For this review, take the finished solid that the model builds, in its own axes (mm). Face numbers are marked on the shaded views. A direction names the side the tool comes from. Round coordinates to 2 decimals unless told otherwise and drop trailing zeros. Write each loop counter-clockwise with the first axis right and the second up, starting at its lowest first coordinate (ties: lowest second). Pieces come first, ordered by that corner, then holes.
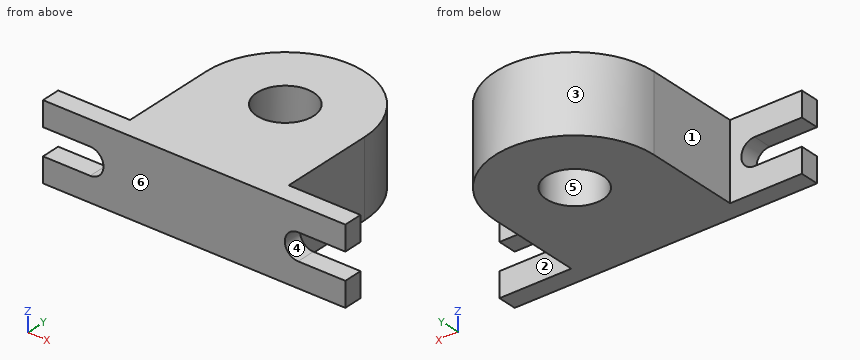
from build123d import *

# Parameters (mm, degrees)
SKETCH_1_R          = 7.5
EXTRUDE_1_DEPTH     = 20
CUT_EXTRUDE_1_DEPTH = 65.156059729


with BuildPart() as part:
    # 草图1 → 凸台-拉伸1 (new body)
    with BuildSketch(Plane.XY):
        with BuildLine():
            Line((21, 0), (21, -25))
            Line((21, -25), (40, -25))
            Line((40, -25), (40, -30))
            Line((40, -30), (21, -30))
            Line((21, -30), (-21, -30))
            Line((-21, -30), (-40, -30))
            Line((-40, -30), (-40, -25))
            Line((-40, -25), (-21, -25))
            Line((-21, -25), (-21, 0))
            ThreePointArc((-21, 0), (0, 21), (21, 0))
        make_face()
        Circle(SKETCH_1_R, mode=Mode.SUBTRACT)
    extrude(amount=EXTRUDE_1_DEPTH)

    # 草图2 → 切除-拉伸1 (cut, through all)
    with BuildSketch(Plane(origin=(0, -25, 0), x_dir=(1, 0, 0), z_dir=(0, 1, 0))):
        with BuildLine():
            Line((-27.5, -6.5), (-40, -6.5))
            Line((-40, -6.5), (-40, -13.5))
            Line((-40, -13.5), (-27.5, -13.5))
            ThreePointArc((-27.5, -13.5), (-24, -10), (-27.5, -6.5))
        make_face()
        with BuildLine():
            Line((40, -13.5), (27.5, -13.5))
            ThreePointArc((27.5, -13.5), (24, -10), (27.5, -6.5))
            Line((27.5, -6.5), (40, -6.5))
            Line((40, -6.5), (40, -13.5))
        make_face()
    extrude(amount=-CUT_EXTRUDE_1_DEPTH, mode=Mode.SUBTRACT)


solid = part.part
(1) We need section A-A, the plane x = 0. Give the boundary of the cut face in (y, z).
Geometry check:
outline: (-30, 0) - (-7.5, 0) - (-7.5, 20) - (-30, 20) - close; (7.5, 0) - (21, 0) - (21, 20) - (7.5, 20) - close
(2) For the marked faces 1, 2 and 3, list the 3-axis set-ups (+Z, -Z, +X, -X, +Y, -Y) from which the entire face can be reached by the end or side of a thin tool; tool diameter is ignored.
Geometry check:
face 1: +Z, -Z, -X, +Y
face 2: +Z, -Z, +X, +Y
face 3: +Z, -Z, +Y
(3) For pin 1 Ø12 at (y, z) = (-2, 16) entering from -X; pin 2 Ø5 at (x, z) = (1.5, 6.5) entering from +Y; pin 3 Ø4 at (x, y) = (-32.5, -26.5) entering from -Z; pin 4 Ø2 at (y, z) = (-10.5, 17.5) entering from +X, all flat-tipped, find the tip position at first contact; note any pin that passes through.
Geometry check:
pin 1: stops at x = -21
pin 2: stops at y = 21
pin 3: stops at z = 0
pin 4: stops at x = 21
(4) We need section B-B, the plane z = 15.25. Give the boundary of the cut face in (x, y), and give its area (3 significant figures).
Geometry check:
outline: (-40, -30) - (40, -30) - (40, -25) - (21, -25) - (21, 0) arc R21 ccw to (-21, 0) - (-21, -25) - (-40, -25) - close; hole circle Ø15 at (0, 0)
area: 1,970 mm2
(5) Mouldability with a two-part tool opening along X and no side actions: class the marked faces 4, 5 and 6 as pulls with the +X half, pulls with the -X half, needs draft (parallel to the pull), parting line crosses it, or undercut.
Geometry check:
face 4: pulls with the +X half
face 5: undercut
face 6: needs draft
(6) We need section C-C, the plane y = -2.5. Give the boundary of the cut face in (x, z), and give its area (3 significant figures).
Geometry check:
outline: (-21, 0) - (-7.07, 0) - (-7.07, 20) - (-21, 20) - close; (7.07, 0) - (21, 0) - (21, 20) - (7.07, 20) - close
area: 557 mm2
(7) We need section D-D, the plane y = -9.5. Give the boundary of the cut face in (x, z).
Geometry check:
outline: (-21, 0) - (21, 0) - (21, 20) - (-21, 20) - close
(8) For line 1 along Y through (x, z) = (0, 5); line 2 along Y through (x, z) = (26, 5.75); line 3 along X through (y, z) = (5.5, 4.5), list the stretches that pass through material, from the lowest coordinate up.
Geometry check:
line 1: y = -30 to -7.5, 7.5 to 21
line 2: y = -30 to -25
line 3: x = -20.27 to -5.1, 5.1 to 20.27
